```python
from build123d import *

# Parameters (mm, degrees)
BOSS_EXTRUDE1_DEPTH                      = 30
SKETCH2_W                                = 30
SKETCH2_H                                = 30
BOSS_EXTRUDE2_DEPTH                      = 10
SKETCH3_R                                = 65
BOSS_EXTRUDE3_DEPTH                      = 3.01
SKETCH4_R                                = 30
BOSS_EXTRUDE4_DEPTH                      = 8
CBORE_FOR_M6_PAN_HEAD_SCREW1_D           = 7
CBORE_FOR_M6_PAN_HEAD_SCREW1_DEPTH       = 50.5
CBORE_FOR_M6_PAN_HEAD_SCREW1_CBORE_D     = 13
CBORE_FOR_M6_PAN_HEAD_SCREW1_CBORE_DEPTH = 4.6
CBORE_FOR_M6_PAN_HEAD_SCREW1_TIP         = 2.103012167


with BuildPart() as part:
    # Sketch1 → Boss-Extrude1 (new body)
    with BuildSketch(Plane(origin=(0, 0, 0), x_dir=(1, 0, 0), z_dir=(0, 1, 0))):
        with BuildLine():
            Line((11.612208492, 155.9994544), (-73.209898492, 176.956548554))
            ThreePointArc((-73.209898492, 176.956548554), (-160, 109), (-73.209898492, 41.043451446))
            Line((-73.209898492, 41.043451446), (11.610000013, 61.999999948))
            Line((11.610000013, 61.999999948), (11.612208492, 62.0005456))
            ThreePointArc((11.612208492, 62.0005456), (48.412726633, 109), (11.612208492, 155.9994544))
        make_face()
    extrude(amount=BOSS_EXTRUDE1_DEPTH)

    # Sketch2 → Boss-Extrude2 (add)
    with BuildSketch(Plane(origin=(0, 30, 0), x_dir=(1, 0, 0), z_dir=(0, 1, 0))):
        with Locations((-90, 109)):
            Rectangle(SKETCH2_W, SKETCH2_H)
    extrude(amount=BOSS_EXTRUDE2_DEPTH)

    # Sketch3 → Boss-Extrude3 (add)
    with BuildSketch(Plane.XZ):
        with Locations(Location((-90, -109, 0), (0, 0, 90))):
            Circle(SKETCH3_R)
    extrude(amount=BOSS_EXTRUDE3_DEPTH)

    # Sketch4 → Boss-Extrude4 (add)
    with BuildSketch(Plane.XZ.offset(3.01)):
        with Locations(Location((-90, -109, 0), (0, 0, 270))):
            Circle(SKETCH4_R)
    extrude(amount=BOSS_EXTRUDE4_DEPTH)

    # CBORE for M6 Pan Head Screw1
    with Locations(Plane(origin=(11.612208492, 0, -79), x_dir=(0, 0, -1), z_dir=(0, -1, 0))):
        with Locations((0, 0), (60, 0)):
            CounterBoreHole(CBORE_FOR_M6_PAN_HEAD_SCREW1_D / 2, CBORE_FOR_M6_PAN_HEAD_SCREW1_CBORE_D / 2, CBORE_FOR_M6_PAN_HEAD_SCREW1_CBORE_DEPTH, depth=CBORE_FOR_M6_PAN_HEAD_SCREW1_DEPTH)
            with Locations((0, 0, -(CBORE_FOR_M6_PAN_HEAD_SCREW1_DEPTH + CBORE_FOR_M6_PAN_HEAD_SCREW1_TIP / 2))):  # 118° drill point
                Cone(0, CBORE_FOR_M6_PAN_HEAD_SCREW1_D / 2, CBORE_FOR_M6_PAN_HEAD_SCREW1_TIP, mode=Mode.SUBTRACT)


solid = part.part
```
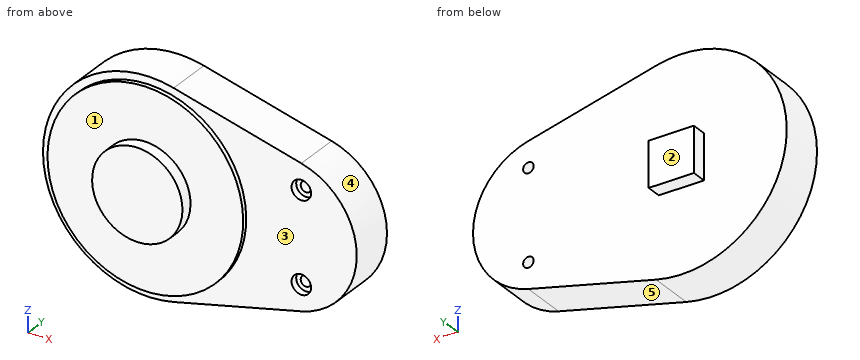
Here's how the part is built. I have some questions about the finished solid (model axes, mm). Face numbers are marked on the shaded views. A direction names the side the tool comes from. Coordinates: 2 decimals unless noted, no trailing zeros. Order: outer loops, then holes, each group sorted by start corner. A loop starts at its lowest first (then second) coordinate and runs counter-clockwise, first axis right, second up. Notation, with made-up numbers: (-29.75, 37.5) - (0.25, 37.5) arc R12 ccw to (0.25, 49.5) - close; hole circle Ø5 at (-27.75, 55.25). An arc over 180 degrees is marked (long way). One line per question, with ' | ' between items. Start each with the question number.
1. If we section it at B-B (x = -90): Write out the boundary of the cut face in (y, z), and give its area (3 significant figures).
2. If we section it at D-D (y = 34): Write out the boundary of the cut face in (x, z), and give its area (3 significant figures).
3. Which directions (+Z, -Z, +X, -X, +Y, -Y) give clear straight access to the entire face, cutting with the end or side of a thin tool? Please do the marked faces 1 and 2.
4. If we mould it in two halves opening along Z, with no side actions, what happens to the marked faces 3, 4 and 5? For each: released by +Z, released by -Z, zero draft, split by the parting line, or undercut.
5. Please list where these lines run through material, in increasing order: line 1 along Y through (x, z) = (-78.5, -62.5); line 2 along Y through (x, z) = (21, -128); line 3 along X through (y, z) = (4.5, -110.5). Write a range as [from, to].
6. If we section it at A-A (y = 11): Give the number of separate pieces and of enclosed holes in the cut face, and give its area (3 significant figures).
7. I'm going to push flat-ended pins straight in: pin 1 Ø6 at (y, z) = (31.5, -111) entering from -X; pin 2 Ø1 at (x, z) = (-17.5, -127.5) entering from +Y; pin 3 Ø4 at (x, z) = (10, -79.5) entering from -Y. Where does each tip first touch, or does it pass through?
8. If we section it at C-C (z = -50): Write out the boundary of the cut face in (x, y).
Model answer:
1) outline: (-11.01, -139) - (-3.01, -139) - (-3.01, -174) - (0, -174) - (0, -179) - (30, -179) - (30, -124) - (40, -124) - (40, -94) - (30, -94) - (30, -39) - (0, -39) - (0, -44) - (-3.01, -44) - (-3.01, -79) - (-11.01, -79) - close | area: 5,370 mm²
2) outline: (-105, -124) - (-75, -124) - (-75, -94) - (-105, -94) - close | area: 900 mm²
3) face 1: -Y | face 2: +Z, -Z, +X, -X, +Y
4) face 3: zero draft | face 4: split by the parting line | face 5: released by -Z
5) line 1: y = [-3.01, 30] | line 2: y = [0, 30] | line 3: x = [-159.98, 48.39]
6) separate pieces: 1 | enclosed holes: 2 | area: 22,300 mm²
7) pin 1: stops at x = -160 | pin 2: stops at y = 30 | pin 3: stops at y = 4.6
8) outline: (-127.67, 0) - (-117.28, 0) - (-117.28, -3.01) - (-62.72, -3.01) - (-62.72, 0) - (-36.96, 0) - (-36.96, 30) - (-127.67, 30) - close
